from build123d import *

# Parameters (mm, degrees)
SKETCH_1_W          = 70
SKETCH_1_H          = 70
SKETCH_1_R          = 6
EXTRUDE_1_DEPTH     = 10
SKETCH_2_W          = 70
SKETCH_2_H          = 5
EXTRUDE_2_DEPTH     = 100
SKETCH_4_R          = 12.5
CUT_EXTRUDE_1_DEPTH = 10


with BuildPart() as part:
    # 草图1 → 凸台-拉伸1 (new body)
    with BuildSketch(Plane.XY):
        with Locations((20, 20)):
            Rectangle(SKETCH_1_W, SKETCH_1_H)
        Circle(SKETCH_1_R, mode=Mode.SUBTRACT)
        with Locations((0, 30)):
            Circle(SKETCH_1_R, mode=Mode.SUBTRACT)
        with Locations((40, 30)):
            Circle(SKETCH_1_R, mode=Mode.SUBTRACT)
        with Locations((40, 0)):
            Circle(SKETCH_1_R, mode=Mode.SUBTRACT)
    extrude(amount=EXTRUDE_1_DEPTH)

    # 草图2 → 凸台-拉伸2 (add)
    with BuildSketch(Plane.XY.offset(10)):
        with Locations((20, 57.5)):
            Rectangle(SKETCH_2_W, SKETCH_2_H)
    extrude(amount=-EXTRUDE_2_DEPTH)

    # 草图4 → 切除-拉伸1 (cut)
    with BuildSketch(Plane(origin=(0, 60, 0), x_dir=(1, 0, 0), z_dir=(0, 1, 0))):
        with Locations(Location((20, 65, 0), (0, 0, 270))):
            Circle(SKETCH_4_R)
        with BuildLine():
            Line((-5, 65), (-5, 0))
            Line((-5, 0), (-73.267990544, 0))
            Line((-73.267990544, 0), (-73.267990544, 50))
            Line((-73.267990544, 50), (-73.267990544, 103.705684911))
            Line((-73.267990544, 103.705684911), (78.593427938, 103.705684911))
            Line((78.593427938, 103.705684911), (78.593427938, 0))
            Line((78.593427938, 0), (45, 0))
            Line((45, 0), (45, 65))
            ThreePointArc((45, 65), (20, 90), (-5, 65))
        make_face()
    extrude(amount=-CUT_EXTRUDE_1_DEPTH, mode=Mode.SUBTRACT)


solid = part.part
Check sheet for the modelled part. Datum: model origin and axes. Units: mm. A direction names the side the tool comes from. Coordinates: 2 decimals unless noted, no trailing zeros. Write each loop counter-clockwise with the first axis right and the second up, starting at its lowest first coordinate (ties: lowest second). Pieces come first, ordered by that corner, then holes.
Item 1: Cross-section at D-D on z = -43.5. Record the boundary of the cut face in (x, y).
Numbers:
outline: (-5, 55) - (45, 55) - (45, 60) - (-5, 60) - close
Item 2: Mould release check, pull along Y, two halves, no side actions. Record for faces 4 (the face through (20, 55, -34)), 5 (the face through (34, 0, 5)), 6 (the face through (20.55, 57.535, -89.994)), 7 (the face through (20, 60, -28)): released by +Y, released by -Y, zero draft, split by the parting line, or undercut.
Numbers:
face 4: released by -Y
face 5: undercut
face 6: zero draft
face 7: released by +Y
Item 3: Access from +Z, -Z, +X, -X, +Y, -Y to the whole of each face (thin tool, end or side, straight path). Record for faces 1 (the face through (-5, 58, -33)), 2 (the face through (55, 22, 5)), 3 (the face through (45, 58, -32)).
Numbers:
face 1: -Z, -X, +Y, -Y
face 2: +Z, -Z, +X, +Y, -Y
face 3: -Z, +X, +Y, -Y
Item 4: Cross-section at B-B on x = 20. Record the boundary of the cut face in (y, z), then the cut area to 4 significant figures.
Numbers:
outline: (-15, 0) - (55, 0) - (55, -52.5) - (60, -52.5) - (60, 10) - (-15, 10) - close; (55, -90) - (60, -90) - (60, -77.5) - (55, -77.5) - close
area: 1,075 mm2
Item 5: Depth check by flat-ended pin: pin 1 Ø5.5 at (y, z) = (58.5, -32.5) entering from -X; pin 2 Ø7 at (x, y) = (0, 0) entering from -Z; pin 3 Ø1.5 at (y, z) = (57.5, -24) entering from +X; pin 4 Ø4 at (x, z) = (30, -61) entering from -Y. Enter the tip coordinate at first touch or a pass-through.
Numbers:
pin 1: stops at x = -5
pin 2: passes through
pin 3: stops at x = 45
pin 4: stops at y = 55
Item 6: Scan lines: probe 1 along Y at (x, z) = (0, 7.5); probe 2 along X at (y, z) = (56, -65); probe 3 along Z at (x, y) = (41.5, 20.5). Record each from-to range of solid material in increasing order.
Numbers:
probe 1: y = -15 to -6, 6 to 24, 36 to 60
probe 2: x = -5 to 7.5, 32.5 to 45
probe 3: z = 0 to 10
Item 7: Cross-section at A-A on y = 0. Record the boundary of the cut face in (x, z).
Numbers:
outline: (-15, 0) - (-6, 0) - (-6, 10) - (-15, 10) - close; (6, 0) - (34, 0) - (34, 10) - (6, 10) - close; (46, 0) - (55, 0) - (55, 10) - (46, 10) - close
Item 8: Cross-section at C-C on x = 40. Record the boundary of the cut face in (y, z), then the cut area to 3 significant figures.
Numbers:
outline: (-15, 0) - (-6, 0) - (-6, 10) - (-15, 10) - close; (6, 0) - (24, 0) - (24, 10) - (6, 10) - close; (36, 0) - (55, 0) - (55, -80) - (60, -80) - (60, 10) - (36, 10) - close
area: 910 mm2
